Here's how the part is built. I have some questions about the finished solid (model axes, mm). Face numbers are marked on the shaded views. A direction names the side the tool comes from. Coordinates: 2 decimals unless noted, no trailing zeros. Loops run counter-clockwise (first coordinate to the right, second up) from the corner with the lowest first, then second, coordinate; pieces in that order, holes last. Notation, with made-up numbers: (14, -26) -> (52, -26) arc R24 ccw to (52, 10) -> close; hole circle Ø8 at (55.5, 89.5). An arc over 180 degrees is marked (long way). Answer as a JSON object with one key per item and string values. Group by question number.
1) Which directions (+Z, -Z, +X, -X, +Y, -Y) give clear straight access to the entire face, cutting with the end or side of a thin tool? Please do the marked faces 1, 2, 3 and 4.
2) I want a section at A-A (y = 8.5). Write out the boundary of the cut face in (x, z), then the cut area to 3 significant figures.
3) If we mould it in two halves opening along X, with no side actions, what happens to the marked faces 5, 6 and 7? For each: +X half, -X half, draft (parallel to the pull), parting line (faces both ways), or undercut.
4) I want a section at B-B (y = 17). Write out the boundary of the cut face in (x, z).
5) I need wall thicknesses on probe 1 along X at (y, z) = (26.35, 0); probe 2 along Y at (x, z) = (26.5, 47); probe 3 along X at (y, z) = (7, 0). Which ranges of each line are inside material? Lowest first, please. Write a range as [from, to].
6) I'm going to push flat-ended pins straight in: pin 1 (1 mm diameter, centred on y = -12.5, z = -16.5, fed in from +X); pin 2 (1 mm diameter, centred on x = -38, z = 34.5, fed in from +Y); pin 3 (12 mm diameter, centred on y = 14, z = -43.5, fed in from -X); pin 4 (20 mm diameter, centred on x = 0, z = 0, fed in from +Y). Where does each tip first touch, or does it pass through?
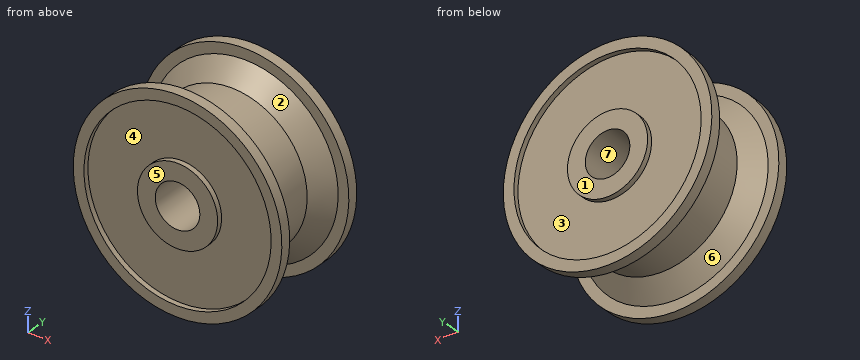
```python
from build123d import *

# Parameters (mm, degrees)
SKETCH_2_R          = 12.5
CUT_EXTRUDE_1_DEPTH = 101.466412298
SKETCH_3_R          = 52.5
SKETCH_3_R_2        = 22.5
CUT_EXTRUDE_2_DEPTH = 3


with BuildPart() as part:
    # 草图1 → 旋转1 (revolve)
    with BuildSketch(Plane.XY, mode=Mode.PRIVATE) as revolve_1_sk:
        Polygon((52.5, 22.5), (58.5, 22.5), (58.5, 28.5), (0, 28.5), (0, -28.5), (58.5, -28.5), (58.5, -22.5), (52.5, -22.5), (42.5, -12.5), (42.5, 12.5), align=None)
    revolve(revolve_1_sk.sketch.rotate(Axis((0, -28.5, 0), (0, 1, 0)), 90), axis=Axis((0, -28.5, 0), (0, 1, 0)))

    # 草图2 → 切除-拉伸1 (cut, through all)
    with BuildSketch(Plane.XZ.offset(28.5)):
        with Locations(Location((0, 0, 0), (0, 0, 270))):
            Circle(SKETCH_2_R)
    extrude(amount=-CUT_EXTRUDE_1_DEPTH, mode=Mode.SUBTRACT)

    # 草图3 → 切除-拉伸2 (cut)
    with BuildSketch(Plane.XZ.offset(28.5)):
        with Locations(Location((0, 0, 0), (0, 0, 270))):
            Circle(SKETCH_3_R)
        with Locations(Location((0, 0, 0), (0, 0, 270))):
            Circle(SKETCH_3_R_2, mode=Mode.SUBTRACT)
    cut_extrude_2 = extrude(amount=-CUT_EXTRUDE_2_DEPTH, mode=Mode.SUBTRACT)

    # 镜向1: 切除-拉伸2 across plane
    add(cut_extrude_2.mirror(Plane.ZX), mode=Mode.SUBTRACT)


solid = part.part
```
Determined:
{
 "1": {"face 1": "+Z, -Z, +X, -X, +Y", "face 2": "none", "face 3": "+Y", "face 4": "-Y"},
 "2": {"outline": "circle Ø85 at (0, 0); hole circle Ø25 at (0, 0)", "area": "5,180 mm^2"},
 "3": {"face 5": "draft", "face 6": "parting line", "face 7": "undercut"},
 "4": {"outline": "circle Ø94 at (0, 0); hole circle Ø25 at (0, 0)"},
 "5": {"probe 1": "[-58.5, -52.5], [-22.5, -12.5], [12.5, 22.5], [52.5, 58.5]", "probe 2": "[-28.5, -22.5], [22.5, 28.5]", "probe 3": "[-42.5, -12.5], [12.5, 42.5]"},
 "6": {"pin 1": "x = 39.75", "pin 2": "y = 25.5", "pin 3": "x = -28.11", "pin 4": "through"}
}
